```python
from build123d import *

# Parameters (mm, degrees)
SKETCH1_R                = 50
SKETCH1_R_2              = 40
BOSS_EXTRUDE1_DEPTH      = 1049
SKETCH10_R               = 45
CUT_EXTRUDE8_DEPTH       = 12
SKETCH13_R               = 44.375
CUT_EXTRUDE10_DEPTH      = 40
CHAMFER5_SIZE            = 1
SKETCH14_R               = 40.875
CUT_EXTRUDE11_DEPTH      = 40
CUT_EXTRUDE12_DEPTH      = 1052.380521029
CUT_EXTRUDE12_DEPTH_BACK = 1052.380521029
SKETCH15_W               = 6
SKETCH15_H               = 40


with BuildPart() as part:
    # Sketch1 → Boss-Extrude1 (new body)
    with BuildSketch(Plane(origin=(0, 0, 0), x_dir=(1, 0, 0), z_dir=(0, 1, 0))):
        with Locations(Location((0, 0, 0), (0, 0, 270))):
            Circle(SKETCH1_R)
        with Locations(Location((0, 0, 0), (0, 0, 270))):
            Circle(SKETCH1_R_2, mode=Mode.SUBTRACT)
    extrude(amount=BOSS_EXTRUDE1_DEPTH)

    # Sketch10 → Cut-Extrude8 (cut)
    with BuildSketch(Plane(origin=(0, 1049, 0), x_dir=(1, 0, 0), z_dir=(0, 1, 0))):
        with Locations(Location((0, 0, 0), (0, 0, 270))):
            Circle(SKETCH10_R)
    extrude(amount=-CUT_EXTRUDE8_DEPTH, mode=Mode.SUBTRACT)

    # Sketch13 → Cut-Extrude10 (cut)
    with BuildSketch(Plane.XZ):
        with Locations(Location((0, 0, 0), (0, 0, 270))):
            Circle(SKETCH13_R)
    extrude(amount=-CUT_EXTRUDE10_DEPTH, mode=Mode.SUBTRACT)

    # Chamfer5
    chamfer5_edges = [part.edges().sort_by_distance(p)[0] for p in [
        (0, 0, 44.375),
        (0, 0, -50),
    ]]
    chamfer(chamfer5_edges, length=CHAMFER5_SIZE)

    # Sketch14 → Cut-Extrude11 (cut)
    with BuildSketch(Plane(origin=(0, 1037, 0), x_dir=(1, 0, 0), z_dir=(0, 1, 0))):
        with Locations(Location((0, 0, 0), (0, 0, 270))):
            Circle(SKETCH14_R)
    extrude(amount=-CUT_EXTRUDE11_DEPTH, mode=Mode.SUBTRACT)

    # Sketch15 → Cut-Extrude12 (cut, two sides: drawn at the far end of the back side and taken through both)
    with BuildSketch(Plane.XY.offset(-CUT_EXTRUDE12_DEPTH_BACK)):
        with Locations((-50, 1049)):
            Rectangle(SKETCH15_W, SKETCH15_H)
    extrude(amount=CUT_EXTRUDE12_DEPTH + CUT_EXTRUDE12_DEPTH_BACK, mode=Mode.SUBTRACT)


solid = part.part
```
Input: part model. Units: mm. Frame: model coordinates. A direction names the side the tool comes from. Round coordinates to 2 decimals unless told otherwise and drop trailing zeros. Loops run counter-clockwise (first coordinate to the right, second up) from the corner with the lowest first, then second, coordinate; pieces in that order, holes last. Notation, with made-up numbers: (44.25, -4.5) - (75.25, -4.5) arc R23 ccw to (75.25, 16.5) - close; hole circle Ø3 at (-35, 22.5). An arc over 180 degrees is marked (long way). One line per item, written item: value. Start each with the question number.
(1) Draft query along Z for faces 4 (the cylindrical face through (13.329, 20.227, -42.326)), 5 (the cylindrical face through (15.02, 517.66, 47.69)), 6 (the flat face through (-47, 1039, 0)). Return one class per face: +Z half, -Z half, draft (parallel to the pull), parting line (faces both ways), or undercut.
(2) Section A-A, the plane z = 0. Return loops of the section in (x, y) (3 decimals), plus the area to 3 significant figures.
(3) Access query for faces 1 (the flat face through (-43.3, 0, 14.3)), 2 (the flat face through (40, 40, 7)), 3 (the cylindrical face through (-39.903, 1017.28, -8.861)). Directions: +Z, -Z, +X, -X, +Y, -Y. A direction counts if a zero-diameter tool reaches every point of the face in a straight line with its end or side. Return the directions, or none.
(4) Section B-B, the plane x = 0. Return loops of the section in (y, z) (3 decimals), plus the area to 3 significant figures.
(5) Section C-C, the plane y = 836.5. Return loops of the section in (x, z), plus the area to 3 significant figures.
(6) Contact query for flat-ended pins moving along their axis: P1, Ø6, axis at y = 351.5, z = -3.5, coming from the +X side; P2, Ø5, axis at x = 22.5, y = 888.5, coming from the +Z side; P3, Ø1.5, axis at x = 34, y = 719.5, coming from the +Z side. Output: stop coordinate, or through.
(7) Ray query, line 1 (X direction, y = 1044, z = 0); line 2 (X direction, y = 625, z = 0); line 3 (Z direction, x = 23, y = 208). Return the intervals inside material, ascending. Write a range as [from, to].
Results below:
1. face 4: undercut
1. face 5: parting line
1. face 6: draft
2. outline: (-50, 1) - (-49, 0) - (-45.375, 0) - (-44.375, 1) - (-44.375, 40) - (-40, 40) - (-40, 997) - (-40.875, 997) - (-40.875, 1037) - (-45, 1037) - (-45, 1049) - (-47, 1049) - (-47, 1029) - (-50, 1029) - close; (40, 40) - (44.375, 40) - (44.375, 1) - (45.375, 0) - (49, 0) - (50, 1) - (50, 1049) - (45, 1049) - (45, 1037) - (40.875, 1037) - (40.875, 997) - (40, 997) - close
2. area: 20,400 mm^2
3. face 1: +Z, -Z, +X, -X, -Y
3. face 2: -Y
3. face 3: +Y
4. outline: (0, -49) - (1, -50) - (1049, -50) - (1049, -45) - (1037, -45) - (1037, -40.875) - (997, -40.875) - (997, -40) - (40, -40) - (40, -44.375) - (1, -44.375) - (0, -45.375) - close; (0, 45.375) - (1, 44.375) - (40, 44.375) - (40, 40) - (997, 40) - (997, 40.875) - (1037, 40.875) - (1037, 45) - (1049, 45) - (1049, 50) - (1, 50) - (0, 49) - close
4. area: 20,400 mm^2
5. outline: circle Ø100 at (0, 0); hole circle Ø80 at (0, 0)
5. area: 2,830 mm^2
6. P1: x = 50
6. P2: z = 45.83
6. P3: z = 37.34
7. line 1: [-47, -45], [45, 50]
7. line 2: [-50, -40], [40, 50]
7. line 3: [-44.4, -32.73], [32.73, 44.4]
